The drawing under review shows one solid part. Ordinate dimensions are in mm from its lowest x, y, z. Give positions to 0.01 mm unless a question says otherwise; leave off trailing zeros. Loops run counter-clockwise (first coordinate to the right, second up) from the corner with the lowest first, then second, coordinate; pieces in that order, holes last. Notation, with made-up numbers: (62, 33.5) - (87, 33.5) arc R34 ccw to (87, 66.5) - close; hole circle Ø2 at (48.5, -21). An arc over 180 degrees is marked (long way). Write each question's results on one line, items separated by ' | '.
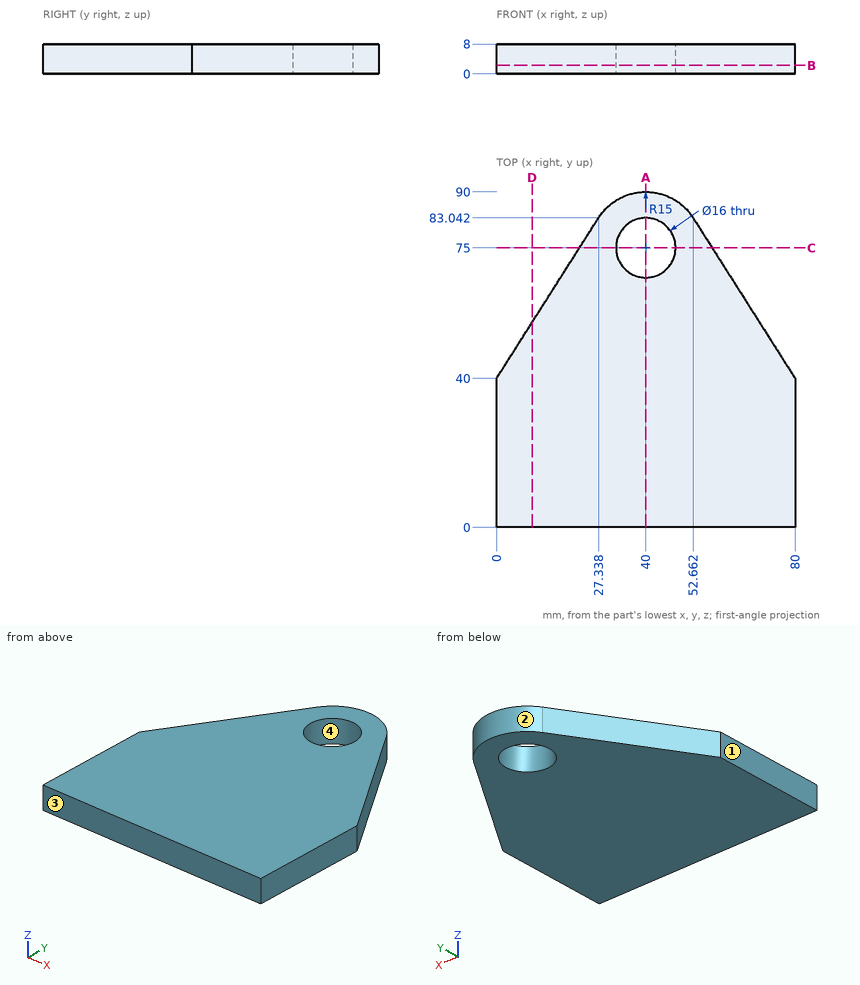
(1) Take a section at C-C on y = 75. Give the boundary of the cut face in (x, z).
Answers below:
outline: (22.23, 0) - (32, 0) - (32, 8) - (22.23, 8) - close; (48, 0) - (57.77, 0) - (57.77, 8) - (48, 8) - close
(2) Take a section at D-D on x = 9.5. Give the boundary of the cut face in (y, z), plus the area to 3 significant figures.
Answers below:
outline: (0, 0) - (54.96, 0) - (54.96, 8) - (0, 8) - close | area: 440 mm2
(3) Take a section at B-B on z = 2.25. Give the boundary of the cut face in (x, y).
Answers below:
outline: (0, 0) - (80, 0) - (80, 40) - (52.66, 83.04) arc R15 ccw to (27.34, 83.04) - (0, 40) - close; hole circle Ø16 at (40, 75)
(4) Wall thickness on line 1 along Y through (x, z) = (40, 5); line 2 along X through (y, z) = (68, 2.75) (1 decimal); line 3 along X through (y, z) = (69, 6.5): over which ranges is each line inside the solid? List them lowest first. Write a range as from..to.
Answers below:
line 1: 0..67, 83..90 | line 2: 17.8..36.1, 43.9..62.2 | line 3: 18.42..34.71, 45.29..61.58
(5) Insertion check: P1, Ø2, axis at x = 15.5, z = 5, coming from the +Y side. The pin has a flat end and moves straight along its axis. Give the tip position at first contact, or say it passes through.
Answers below:
P1: y = 65.98
(6) Draft analysis for pull direction Y (two halves, no side actions). For the marked faces 1, 2, 3 and 4, state which applies: pulls with the +Y half, pulls with the -Y half, needs draft (parallel to the pull), parting line crosses it, or undercut.
Answers below:
face 1: needs draft | face 2: pulls with the +Y half | face 3: pulls with the -Y half | face 4: undercut
(7) Take a section at A-A on x = 40. Give the boundary of the cut face in (y, z).
Answers below:
outline: (0, 0) - (67, 0) - (67, 8) - (0, 8) - close; (83, 0) - (90, 0) - (90, 8) - (83, 8) - close
